```python
from build123d import *


with BuildPart() as part:
    # Pin Profile Sketch → Pin Body Revolve (revolve)
    with BuildSketch(Plane.XY, mode=Mode.PRIVATE) as pin_body_revolve_sk:
        Polygon((0, 0), (12.5, 0), (12.5, 50), (16, 50), (16, 150), (12.5, 150), (12.5, 200), (0, 200), align=None)
    revolve(pin_body_revolve_sk.sketch.rotate(Axis((0, 200, 0), (0, -1, 0)), 180), axis=Axis((0, 200, 0), (0, -1, 0)))


solid = part.part
```
Part model, mm, in its own coordinate system. A direction names the side the tool comes from. Round coordinates to 2 decimals unless told otherwise and drop trailing zeros. Loops run counter-clockwise (first coordinate to the right, second up) from the corner with the lowest first, then second, coordinate; pieces in that order, holes last. Notation, with made-up numbers: (-25.5, 50.5) -> (16.5, 50.5) arc R20 ccw to (16.5, 81.5) -> close; hole circle Ø8 at (30, -11). An arc over 180 degrees is marked (long way). Use one line per item in the form item = value. Start each with the question number.
Item 1: Band-saw the part on C-C (y = 33). List the corners of the cut face in (x, z), plus the area to 3 significant figures.
Item 2: Band-saw the part on A-A (x = 5). List the corners of the cut face in (y, z), plus the area to 3 significant figures.
Item 3: Band-saw the part on D-D (y = 144.5). List the corners of the cut face in (x, z), plus the area to 3 significant figures.
Item 4: Band-saw the part on B-B (z = 8.5). List the corners of the cut face in (x, y), plus the area to 3 significant figures.
Item 5: Drill centre lines: line 1 along X through (y, z) = (167, 0.5); line 2 along Y through (x, z) = (7, -14); line 3 along Z through (x, y) = (-1, 189). Where is each one in solid material? Low to high.
Item 6: Drop flat-ended pins along their axis: pin 1 Ø2 at (y, z) = (28.5, -11) entering from +X; pin 2 Ø10 at (x, y) = (10, 145) entering from +Z; pin 3 Ø2 at (x, y) = (9, 172) entering from -Z. Give the stop position or say it passes through.
Item 7: Tool access for faces 1 (the flat face through (0, 200, 0)), 2 (the cylindrical face through (-11.923, 25.35, -3.755)), 3 (the flat face through (10, 150, 8)): list every direction of +Z, -Z, +X, -X, +Y, -Y with a clear straight run to the whole face (end or side of a thin tool).
Data:
q1.outline = circle Ø25 at (0, 0)
q1.area = 491 mm^2
q2.outline = (0, -11.46) -> (50, -11.46) -> (50, -15.2) -> (150, -15.2) -> (150, -11.46) -> (200, -11.46) -> (200, 11.46) -> (150, 11.46) -> (150, 15.2) -> (50, 15.2) -> (50, 11.46) -> (0, 11.46) -> close
q2.area = 5,330 mm^2
q3.outline = circle Ø32 at (0, 0)
q3.area = 804 mm^2
q4.outline = (-13.56, 50) -> (-9.17, 50) -> (-9.17, 0) -> (9.17, 0) -> (9.17, 50) -> (13.56, 50) -> (13.56, 150) -> (9.17, 150) -> (9.17, 200) -> (-9.17, 200) -> (-9.17, 150) -> (-13.56, 150) -> close
q4.area = 4,540 mm^2
q5.line_1 = -12.49 to 12.49
q5.line_2 = 50 to 150
q5.line_3 = -12.46 to 12.46
q6.pin_1 = 7.5
q6.pin_2 = 15.2
q6.pin_3 = -9.6
q7.face_1 = +Z, -Z, +X, -X, +Y
q7.face_2 = -Y
q7.face_3 = +Y
